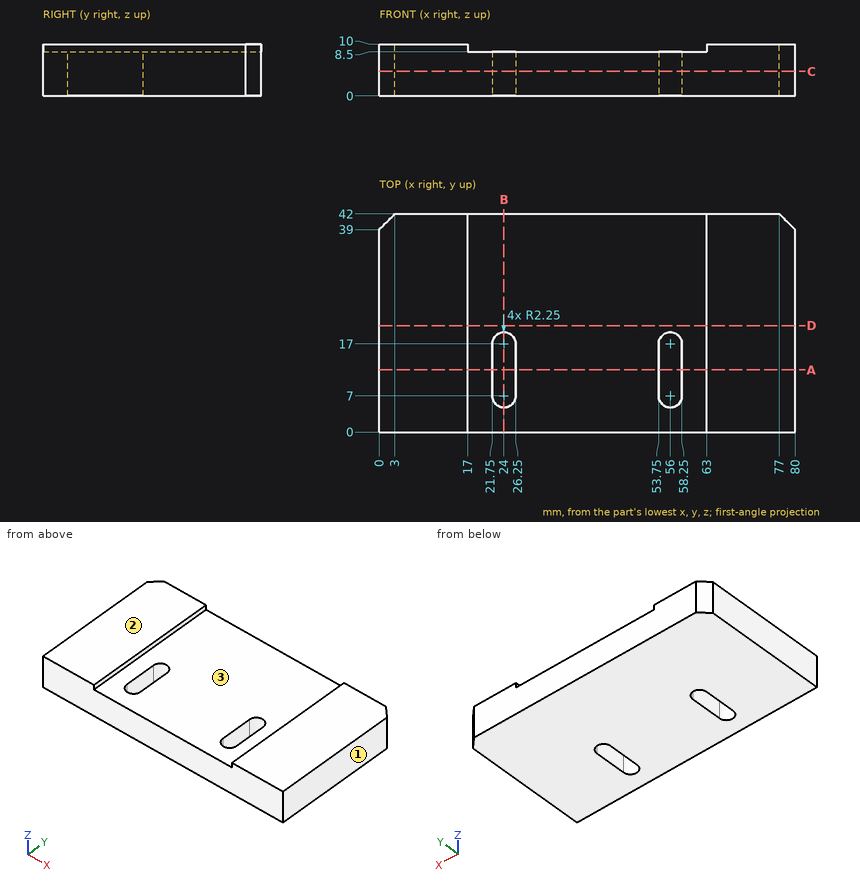
Geometry check sheet. Reference: drawing and pictorial views, mm from the part's lowest x, y, z. Coordinates: 2 decimals unless noted, no trailing zeros. Write each loop counter-clockwise with the first axis right and the second up, starting at its lowest first coordinate (ties: lowest second). Pieces come first, ordered by that corner, then holes. Notation, with made-up numbers: M -7,-32 L 35,-32 A6 ccw 35,-22 Z; hole C 53,-38 d10. An arc over 180 degrees is marked long. Use one line per item in the form item = value.
Item 1: Sectioned sample at C-C, the plane z = 4.75. Record the cut outline in (x, y).
Answer below:
outline = M 0,0 L 80,0 L 80,39 L 77,42 L 3,42 L 0,39 Z; hole M 21.75,7 A2.25 ccw 26.25,7 L 26.25,17 A2.25 ccw 21.75,17 Z; hole M 53.75,7 A2.25 ccw 58.25,7 L 58.25,17 A2.25 ccw 53.75,17 Z
Item 2: Sectioned sample at B-B, the plane x = 24. Record the cut outline in (y, z).
Answer below:
outline = M 0,0 L 4.75,0 L 4.75,8.5 L 0,8.5 Z; M 19.25,0 L 42,0 L 42,8.5 L 19.25,8.5 Z
Item 3: Gauge pin test, flat end, axial feed: pin 1 Ø4 at (y, z) = (11.5, 3) entering from -X. Record the tip position at first contact, or that the pin passes through.
Answer below:
pin_1 = 0
Item 4: Release check for a two-part mould opening along X. For the marked faces 1, 2 and 3 record: pulls with the +X half, pulls with the -X half, needs draft (parallel to the pull), parting line crosses it, or undercut.
Answer below:
face_1 = pulls with the +X half
face_2 = needs draft
face_3 = undercut
Item 5: Sectioned sample at A-A, the plane y = 12. Record the cut outline in (x, z).
Answer below:
outline = M 0,0 L 21.75,0 L 21.75,8.5 L 17,8.5 L 17,10 L 0,10 Z; M 26.25,0 L 53.75,0 L 53.75,8.5 L 26.25,8.5 Z; M 58.25,0 L 80,0 L 80,10 L 63,10 L 63,8.5 L 58.25,8.5 Z
Item 6: Material ranges on L1, parallel to X at y = 10, z = 7.5; L2, parallel to X at y = 28.5, z = 9; L3, parallel to X at y = 6, z = 5.25, recorded low to high. Write a range as from..to.
Answer below:
L1 = 0..21.75, 26.25..53.75, 58.25..80
L2 = 0..17, 63..80
L3 = 0..21.98, 26.02..53.98, 58.02..80
Item 7: Sectioned sample at D-D, the plane y = 20.5. Record the cut outline in (x, z), and give its area (3 significant figures).
Answer below:
outline = M 0,0 L 80,0 L 80,10 L 63,10 L 63,8.5 L 17,8.5 L 17,10 L 0,10 Z
area = 731 mm^2
